The listing builds one solid part. Answer for the finished solid, in the listing's coordinates (mm). Give positions to 0.01 mm unless a question says otherwise; leave off trailing zeros. Write each loop counter-clockwise with the first axis right and the second up, starting at its lowest first coordinate (ties: lowest second). Pieces come first, ordered by that corner, then holes.
```python
from build123d import *

# Parameters (mm, degrees)
SKETCH1_W           = 135
SKETCH1_H           = 220
BOSS_EXTRUDE1_DEPTH = 15
SKETCH2_R           = 11.5
BOSS_EXTRUDE2_DEPTH = 15


with BuildPart() as part:
    # Sketch1 → Boss-Extrude1 (new, symmetric)
    with BuildSketch(Plane.XY):
        Rectangle(SKETCH1_W, SKETCH1_H)
    extrude(amount=BOSS_EXTRUDE1_DEPTH, both=True)

    # Sketch2 → Boss-Extrude2 (add)
    with BuildSketch(Plane(origin=(0, 110, 0), x_dir=(1, 0, 0), z_dir=(0, 1, 0))):
        with Locations((32.5, 0)):
            Circle(SKETCH2_R)
        with Locations((-32.5, 0)):
            Circle(SKETCH2_R)
    extrude(amount=BOSS_EXTRUDE2_DEPTH)


solid = part.part
```
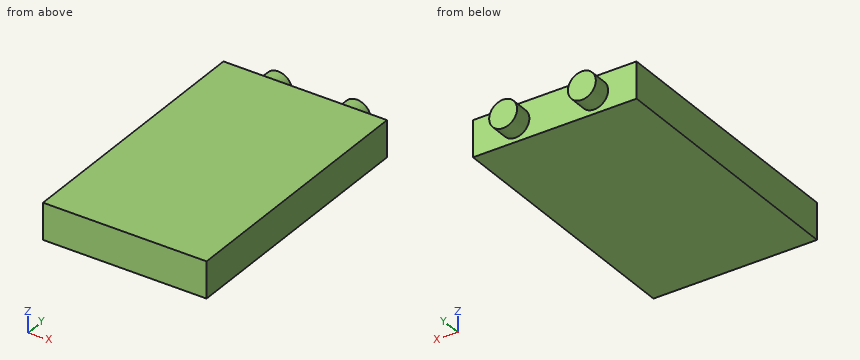
Item 1: A cutting plane is placed at B-B, the plane x = -1. Give the vertices of the cut face in (y, z), plus the area to 3 significant figures.
Conclusion:
outline: (-110, -15) - (110, -15) - (110, 15) - (-110, 15) - close
area: 6,600 mm2
Item 2: A cutting plane is placed at A-A, the plane z = 0. Give the vertices of the cut face in (x, y).
Conclusion:
outline: (-67.5, -110) - (67.5, -110) - (67.5, 110) - (44, 110) - (44, 125) - (21, 125) - (21, 110) - (-21, 110) - (-21, 125) - (-44, 125) - (-44, 110) - (-67.5, 110) - close
Item 3: Consider probe 1 along Y at (x, z) = (18, 1.5); probe 2 along X at (y, z) = (113, -7); probe 3 along Z at (x, y) = (-34.5, 116). Determine where each line is inside the solid, lowest interval first.
Conclusion:
probe 1: y = -110 to 110
probe 2: x = -41.62 to -23.38, 23.38 to 41.62
probe 3: z = -11.32 to 11.32
Item 4: This flat-tipped pin is pushed along its axis until it touches: P1, Ø15, axis at x = -18, z = 2.5, coming from the +Y side. Where does it stop, or does it pass through?
Conclusion:
P1: stops at y = 125
